from build123d import *

# Parameters (mm, degrees)
SKETCH8_R           = 25
SKETCH8_R_2         = 14
BOSS_EXTRUDE2_DEPTH = 4
CUT_EXTRUDE5_REACH  = 92.935
SKETCH9_W           = 8
SKETCH9_H           = 6.6


with BuildPart() as part:
    # Sketch1 → Revolve1 (revolve)
    with BuildSketch(Plane.XY, mode=Mode.PRIVATE) as revolve1_sk:
        Polygon((6.158767395, 41.3), (2.658151092, 52.75), (0, 52.75), (0, 14), (48, 14), (48, 52.75), (45.341848908, 52.75), (41.841232605, 41.3), (36.161232605, 41.3), (32.660616303, 52.75), (30.340616303, 52.75), (26.84, 41.3), (21.16, 41.3), (17.659383697, 52.75), (15.339383697, 52.75), (11.838767395, 41.3), align=None)
    revolve(revolve1_sk.sketch.rotate(Axis((0, 0, 0), (1, 0, 0)), 270), axis=Axis((0, 0, 0), (1, 0, 0)))

    # Sketch8 → Boss-Extrude2 (add)
    with BuildSketch(Plane.ZY):
        Circle(SKETCH8_R)
        with Locations(Location((0, 0, 0), (0, 0, 180))):
            Circle(SKETCH8_R_2, mode=Mode.SUBTRACT)
    extrude(amount=BOSS_EXTRUDE2_DEPTH)

    # Sketch9 → Cut-Extrude5 (cut, up to next)
    with BuildSketch(Plane.ZY.offset(4), mode=Mode.PRIVATE) as cut_extrude5_sk1:
        with Locations((0, 14)):
            Rectangle(SKETCH9_W, SKETCH9_H)
    cut_extrude5_tool1 = extrude(cut_extrude5_sk1.sketch, amount=-CUT_EXTRUDE5_REACH, mode=Mode.PRIVATE) & part.part
    add(cut_extrude5_tool1.solids().sort_by_distance((-4, 14, 0))[0], mode=Mode.SUBTRACT)


solid = part.part
Verification items for the finished model (mm, model axes). A direction names the side the tool comes from. Round coordinates to 2 decimals unless told otherwise and drop trailing zeros. Loops run counter-clockwise (first coordinate to the right, second up) from the corner with the lowest first, then second, coordinate; pieces in that order, holes last. Notation, with made-up numbers: (-3, 17) - (12, 17) arc R28 cw to (12, 52) - close; hole circle Ø1 at (33.5, 55). An arc over 180 degrees is marked (long way). Use a Markdown table: item, result. Add a question column.
1. Thickness scan on probe 1 along X at (y, z) = (-22.5, 36); probe 2 along Y at (x, z) = (7, 0); probe 3 along X at (y, z) = (48.5, 11.5). Record the ranges inside material, lowest first. Write a range as [from, to].
2. Section check A-A, the plane x = 38.5. Record the boundary of the cut face in (y, z).
3. Gauge pin test, flat ends, axial feed: pin 1 (4 mm diameter, centred on x = 25, z = -37, fed in from +Y); pin 2 (1 mm diameter, centred on x = 41, z = -18, fed in from +Y); pin 3 (4 mm diameter, centred on x = 24.5, y = 35, fed in from +Z). Record the tip position at first contact, or that the pin passes through.
4. Section check B-B, the plane z = 43. Give the number of separate pieces and of enclosed holes in the cut face, plus the area to 3 significant figures.
5. Release check for a two-part mould opening along X. For faces 5 (the face through (-4, -11, 11)), 6 (the face through (38.96, 12.41, -39.39)), 7 (the face through (42.01, 12.57, -39.92)), 8 (the face through (22, 17.3, 0)) record: released by +X, released by -X, zero draft, split by the parting line, or undercut.
6. Access from +Z, -Z, +X, -X, +Y, -Y to the whole of each face (thin tool, end or side, straight path). Record for faces 1 (the face through (12.009, 12.572, -39.923)), 2 (the face through (22, 15, -4)), 3 (the face through (48, -11, 11)), 4 (the face through (-1.972, 7.509, 23.846)).
Checks:
| question | item | result |
|---|---|---|
| 1 | probe 1 | x = [0, 5.81], [12.19, 20.81], [27.19, 35.81], [42.19, 48] |
| 1 | probe 2 | y = [-41.3, -14], [17.3, 41.3] |
| 1 | probe 3 | x = [0, 3.55], [14.45, 18.55], [29.45, 33.55], [44.45, 48] |
| 2 | outline | circle Ø82.6 at (0, 0); hole (13.42, -4) - (17.3, -4) - (17.3, 4) - (13.42, 4) arc R14 ccw (long way) to start |
| 3 | pin 1 | stops at y = 21.92 |
| 3 | pin 2 | stops at y = 37.41 |
| 3 | pin 3 | stops at z = 24.83 |
| 4 | separate pieces | 4 |
| 4 | enclosed holes | 0 |
| 4 | area | 1,320 mm^2 |
| 5 | face 5 | released by -X |
| 5 | face 6 | undercut |
| 5 | face 7 | undercut |
| 5 | face 8 | zero draft |
| 6 | face 1 | none |
| 6 | face 2 | +X, -X |
| 6 | face 3 | +Z, -Z, +X, +Y, -Y |
| 6 | face 4 | -X |
